```python
from build123d import *

# Parameters (mm, degrees)
FILLET1_R = 2


with BuildPart() as part:
    # Sketch3 → Revolve1 (revolve)
    with BuildSketch(Plane.XY, mode=Mode.PRIVATE) as revolve1_sk:
        Polygon((0, 0), (0, 12.5), (80, 12.5), (80, 10), (118, 10), (118, 8), (138, 8), (138, 0), align=None)
    revolve(revolve1_sk.sketch.rotate(Axis((0, 0, 0), (1, 0, 0)), 90), axis=Axis((0, 0, 0), (1, 0, 0)))

    # Fillet1
    fillet1_edges = [part.edges().sort_by_distance(p)[0] for p in [
        (0, 0, -12.5),
    ]]
    fillet(fillet1_edges, radius=FILLET1_R)


solid = part.part
```
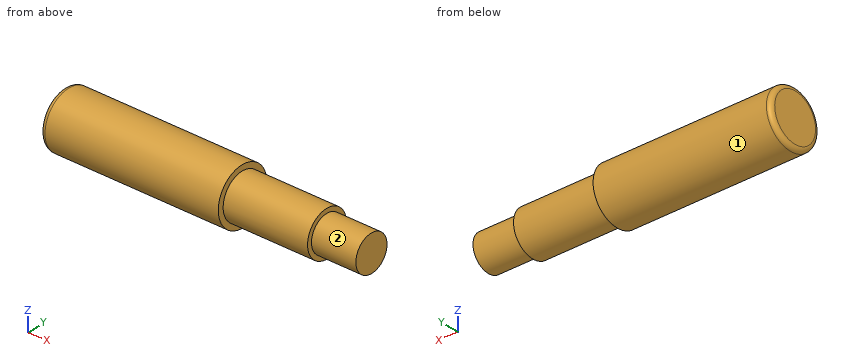
Work out the finished part from the listing and answer in its coordinate system (mm). Face numbers are marked on the shaded views. A direction names the side the tool comes from. Give positions to 0.01 mm unless a question says otherwise; leave off trailing zeros. Write each loop counter-clockwise with the first axis right and the second up, starting at its lowest first coordinate (ties: lowest second). Pieces come first, ordered by that corner, then holes.
(1) The part is cut by section D-D on x = 95. Write down the section's boundary in (y, z), plus the area to 3 significant figures.
Final values:
outline: circle Ø20 at (0, 0)
area: 314 mm2
(2) The part is cut by section A-A on y = 0. Write down the section's boundary in (x, z), plus the area to 3 significant figures.
Final values:
outline: (0, -10.5) arc R2 ccw to (2, -12.5) - (80, -12.5) - (80, -10) - (118, -10) - (118, -8) - (138, -8) - (138, 8) - (118, 8) - (118, 10) - (80, 10) - (80, 12.5) - (2, 12.5) arc R2 ccw to (0, 10.5) - close
area: 3,080 mm2
(3) Which of the six approach directions +Z, -Z, +X, -X, +Y, -Y give full straight-line access (tool end or side, diameter ignored) to the marked faces 1 and 2?
Final values:
face 1: +X, -X
face 2: +X
(4) Straight lines are drawn through the part: line 1 (Z direction, x = 95.5, y = -0.75); line 2 (X direction, y = -2, z = -8); line 3 (Y direction, x = 24.5, z = -6.75). For each, find the intervals that lie inside material, in ascending order.
Final values:
line 1: z = -9.97 to 9.97
line 2: x = 0 to 118
line 3: y = -10.52 to 10.52
(5) The part is cut by section C-C on x = 19.5. Write down the section's boundary in (y, z), plus the area to 3 significant figures.
Final values:
outline: circle Ø25 at (0, 0)
area: 491 mm2
(6) Flat-ended cylindrical pins translate along their axes: pin 1 Ø3 at (y, z) = (9.5, 8.5) entering from -X; pin 2 Ø1.5 at (x, y) = (77.5, 10) entering from -Z; pin 3 Ø1 at (x, y) = (23, 3) entering from +Z. Find the tip coordinate at first contact, or state that the pin passes through.
Final values:
pin 1: stops at x = 0.14
pin 2: stops at z = -8.41
pin 3: stops at z = 12.25
